CAD build for the part. Positions are in the model's coordinates, mm. Face numbers are marked on the shaded views. A direction names the side the tool comes from. Give positions to 0.01 mm unless a question says otherwise; leave off trailing zeros. Loops run counter-clockwise (first coordinate to the right, second up) from the corner with the lowest first, then second, coordinate; pieces in that order, holes last.
Item 1: Saw through at A-A on x = 16.75. Give the cut face in (y, z), plus the area to 3 significant figures.
Item 2: Which spindle directions (+Z, -Z, +X, -X, +Y, -Y) get a long thin tool onto all of the face, cutting with end or side? Do the marked faces 1, 2 and 3. Say none if no direction does.
Item 3: Mould opens along Z. For the marked faces 4, 5 and 6 say: released by +Z, released by -Z, zero draft, split by the parting line, or undercut.
Item 4: Probe probe 1 along Y at (x, z) = (11.5, 0); probe 2 along Y at (x, z) = (2, 2.25); probe 3 along Z at (x, y) = (2.5, 2). List the from-to ranges inside material, lowest first.
Item 5: Drop flat-ended pins along their axis: P1, Ø8, axis at x = 9.5, z = 3, coming from the -Y side; P2, Ø2, axis at x = 11.5, y = -2, coming from the -Z side; P3, Ø1.5, axis at x = 10.5, z = -2.5, coming from the -Y side. Give the stop position or say it passes through.
from build123d import *

# Parameters (mm, degrees)
HEXAGONSOCKET_DEPTH = 3
HEADFILLET_R        = 0.4
CHAMFER_2_SIZE      = 0.6765
SKETCH4_W           = 5
SKETCH4_H           = 5


with BuildPart() as part:
    # Sketch1 → Base (revolve)
    with BuildSketch(Plane.XY, mode=Mode.PRIVATE) as base_sk:
        Polygon((0, 0), (0, 8.96), (4.96, 4), (20, 4), (20, 0), align=None)
    revolve(base_sk.sketch.rotate(Axis((-0.587069181, 0, 0), (1, 0, 0)), 90), axis=Axis((-0.587069181, 0, 0), (1, 0, 0)))

    # Sketch2 → HexagonSocket (cut)
    with BuildSketch(Plane(origin=(0, 0, 0), x_dir=(0, 0, -1), z_dir=(1, 0, 0))):
        Polygon((2.886751346, 0), (1.443375673, 2.5), (-1.443375673, 2.5), (-2.886751346, 0), (-1.443375673, -2.5), (1.443375673, -2.5), align=None)
    extrude(amount=HEXAGONSOCKET_DEPTH, mode=Mode.SUBTRACT)

    # Sketch3 → Cut-Revolve1 (revolve, cut)
    with BuildSketch(Plane.XY, mode=Mode.PRIVATE) as cut_revolve1_sk:
        Polygon((3, 2.5), (4.443375673, 0), (3, 0), align=None)
    revolve(cut_revolve1_sk.sketch.rotate(Axis((-0.439109555, 0, 0), (1, 0, 0)), 90), axis=Axis((-0.439109555, 0, 0), (1, 0, 0)), mode=Mode.SUBTRACT)

    # HeadFillet
    headfillet_edges = [part.edges().sort_by_distance(p)[0] for p in [
        (4.96, 0, -4),
    ]]
    fillet(headfillet_edges, radius=HEADFILLET_R)

    # Chamfer 2
    chamfer_2_edges = [part.edges().sort_by_distance(p)[0] for p in [
        (20, 0, -4),
    ]]
    chamfer(chamfer_2_edges, length=CHAMFER_2_SIZE)

    # Sketch4 → Cut-Revolve2 (revolve, cut)
    with BuildSketch(Plane(origin=(0, 0, 0), x_dir=(1, 0, 0), z_dir=(0, 1, 0)), mode=Mode.PRIVATE) as cut_revolve2_sk:
        with Locations((0.5, 10.12)):
            Rectangle(SKETCH4_W, SKETCH4_H)
    revolve(cut_revolve2_sk.sketch.rotate(Axis((11.853138686, 0, 0), (-1, 0, 0)), 180), axis=Axis((11.853138686, 0, 0), (-1, 0, 0)), mode=Mode.SUBTRACT)


solid = part.part
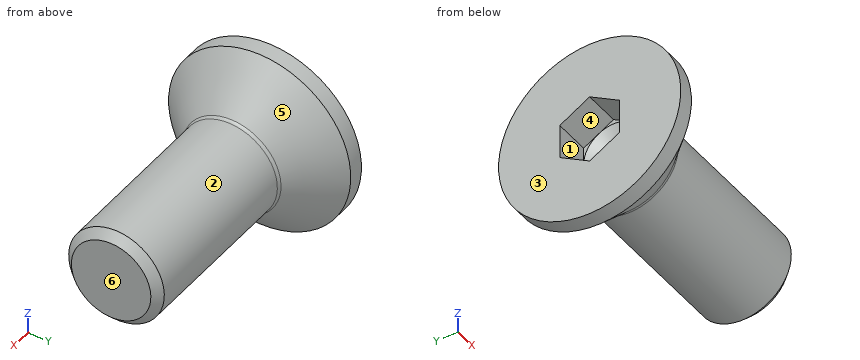
Results below:
1. outline: circle Ø8 at (0, 0)
1. area: 50.3 mm2
2. face 1: -X
2. face 2: +X
2. face 3: +Z, -Z, -X, +Y, -Y
3. face 4: undercut
3. face 5: split by the parting line
3. face 6: zero draft
4. probe 1: y = -4 to 4
4. probe 2: y = -6.59 to -1.1, 1.1 to 6.59
4. probe 3: z = -6.14 to -1.73, 1.73 to 6.14
5. P1: stops at y = -4
5. P2: stops at z = -3.87
5. P3: stops at y = -3.6
